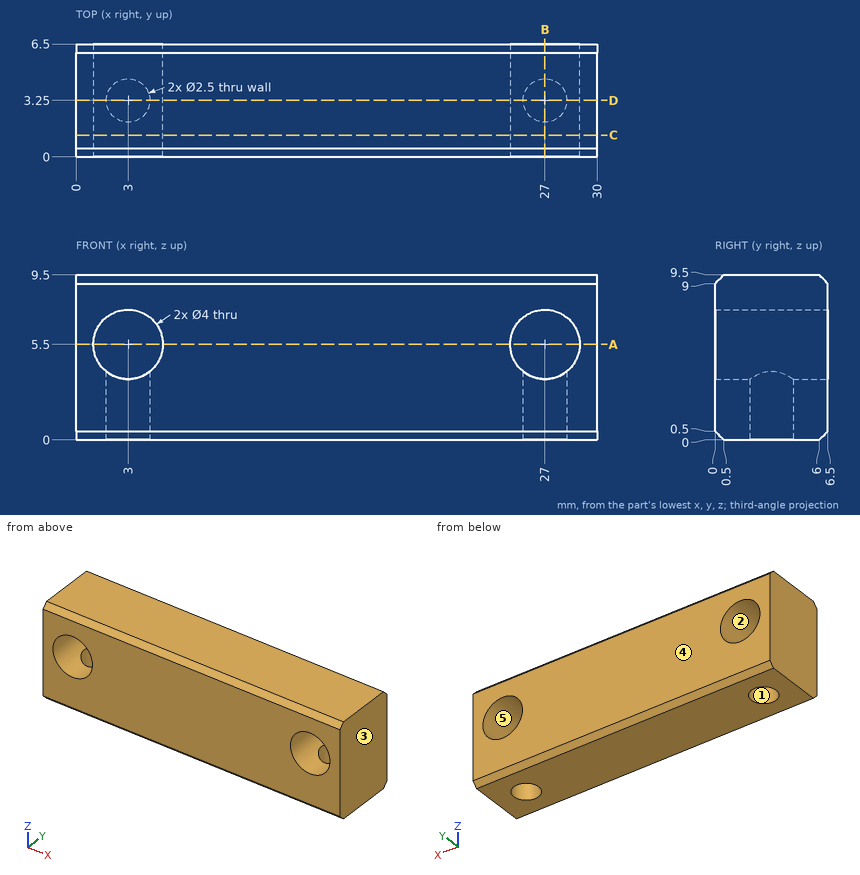
Input: dimensioned drawing with shaded views. Units: mm. Origin: part minimum x, y, z. A direction names the side the tool comes from. Round coordinates to 2 decimals unless told otherwise and drop trailing zeros. Loops run counter-clockwise (first coordinate to the right, second up) from the corner with the lowest first, then second, coordinate; pieces in that order, holes last. Notation, with made-up numbers: (35.5, -39.75) -> (77.5, -39.75) arc R22 ccw to (77.5, -11.75) -> close; hole circle Ø11 at (22.5, 64.5). An arc over 180 degrees is marked (long way). Answer as a JSON object with one key per item and string values. Group by question number.
Q1. Ray query, line 1 (X direction, y = 2.75, z = 2.5); line 2 (Y direction, x = 27, z = 2.35); line 3 (X direction, y = 2.5, z = 3.5). Return the intervals inside material, ascending. Write a range as from..to.
Q2. Contact query for a flat-ended pin moving along its axis: P1, Ø2, axis at x = 27, y = 3.25, coming from the -Z side. Output: stop coordinate, or through.
Q3. Access query for the marked faces 1 and 2. Directions: +Z, -Z, +X, -X, +Y, -Y. A direction counts if a zero-diameter tool reaches every point of the face in a straight line with its end or side. Return the directions, or none.
Q4. Section query C-C (y = 1.25). Output: boundary loops of the cut face in (x, z).
Q5. Mould query, pull axis X, two halves, no side actions, for the marked faces 3, 4 and 5. Classes: pulls with the +X half, pulls with the -X half, needs draft (parallel to the pull), parting line crosses it, or undercut.
Q6. Section query A-A (z = 5.5). Output: boundary loops of the cut face in (x, y), plus the area to 3 significant figures.
Q7. Section query B-B (x = 27). Output: boundary loops of the cut face in (y, z), plus the area to 3 significant figures.
Q8. Section query D-D (y = 3.25). Output: boundary loops of the cut face in (x, z), plus the area to 3 significant figures.
Completed:
{
 "1": {"line 1": "0..1.85, 4.15..25.85, 28.15..30", "line 2": "0..2, 4.5..6.5", "line 3": "0..2, 4..26, 28..30"},
 "2": {"P1": "z = 7.23"},
 "3": {"face 1": "-Z", "face 2": "+Y, -Y"},
 "4": {"outline": "(0, 0) -> (30, 0) -> (30, 9.5) -> (0, 9.5) -> close; hole circle Ø4 at (3, 5.5); hole circle Ø4 at (27, 5.5)"},
 "5": {"face 3": "pulls with the +X half", "face 4": "needs draft", "face 5": "undercut"},
 "6": {"outline": "(0, 0) -> (1, 0) -> (1, 6.5) -> (0, 6.5) -> close; (5, 0) -> (25, 0) -> (25, 6.5) -> (5, 6.5) -> close; (29, 0) -> (30, 0) -> (30, 6.5) -> (29, 6.5) -> close", "area": "143 mm²"},
 "7": {"outline": "(0, 0.5) -> (0.5, 0) -> (2, 0) -> (2, 3.5) -> (0, 3.5) -> close; (0, 7.5) -> (6.5, 7.5) -> (6.5, 9) -> (6, 9.5) -> (0.5, 9.5) -> (0, 9) -> close; (4.5, 0) -> (6, 0) -> (6.5, 0.5) -> (6.5, 3.5) -> (4.5, 3.5) -> close", "area": "26.5 mm²"},
 "8": {"outline": "(0, 0) -> (1.75, 0) -> (1.75, 3.94) arc R2 cw (long way) to (4.25, 3.94) -> (4.25, 0) -> (25.75, 0) -> (25.75, 3.94) arc R2 cw (long way) to (28.25, 3.94) -> (28.25, 0) -> (30, 0) -> (30, 9.5) -> (0, 9.5) -> close", "area": "242 mm²"}
}
